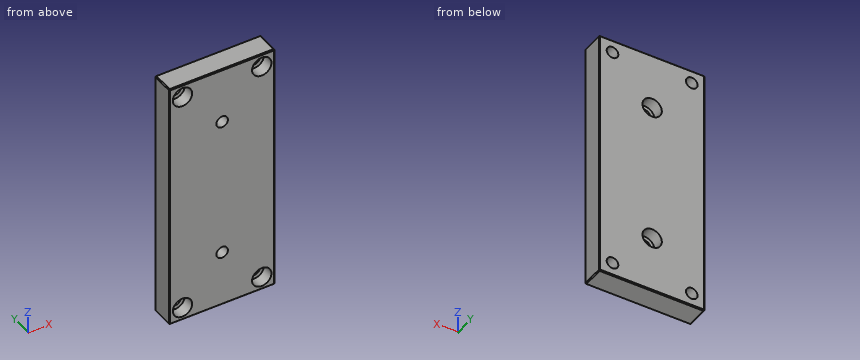
```python
from build123d import *

# Parameters (mm, degrees)
SKETCH_1_W                  = 60
SKETCH_1_H                  = 13
EXTRUDE_1_DEPTH             = 144
HOLE_WIZARD_2_D             = 6.6
HOLE_WIZARD_2_CBORE_D       = 11
HOLE_WIZARD_2_CBORE_DEPTH   = 6.8
CHAMFER_1_SIZE              = 0.5
HOLE_WIZARD_2_2_D           = 6.6
HOLE_WIZARD_2_2_CBORE_D     = 11
HOLE_WIZARD_2_2_CBORE_DEPTH = 6.8


with BuildPart() as part:
    # 草图1 → 凸台-拉伸1 (new body)
    with BuildSketch(Plane.XY):
        Rectangle(SKETCH_1_W, SKETCH_1_H)
    extrude(amount=EXTRUDE_1_DEPTH)

    # Hole Wizard 2 (through all)
    with Locations(Plane(origin=(0, 6.5, 0), x_dir=(1, 0, 0), z_dir=(0, 1, 0))):
        with Locations((0, -32), (0, -112)):
            CounterBoreHole(HOLE_WIZARD_2_D / 2, HOLE_WIZARD_2_CBORE_D / 2, HOLE_WIZARD_2_CBORE_DEPTH)

    # 倒角1
    chamfer_1_edges = [part.edges().sort_by_distance(p)[0] for p in [
        (-30, 0, 144),
        (0, -6.5, 144),
        (30, 0, 144),
        (0, -6.5, 0),
        (-30, 0, 0),
        (0, 6.5, 0),
        (30, 0, 0),
        (0, 6.5, 144),
        (30, -6.5, 72),
        (-30, -6.5, 72),
        (-30, 6.5, 72),
        (30, 6.5, 72),
    ]]
    chamfer(chamfer_1_edges, length=CHAMFER_1_SIZE)

    # Hole Wizard 2 2 (through all)
    with Locations(Plane(origin=(0, -6.5, 0), x_dir=(-1, 0, 0), z_dir=(0, -1, 0))):
        with Locations((-22.5, -136.5), (22.5, -136.5), (-22.5, -7.5), (22.5, -7.5)):
            CounterBoreHole(HOLE_WIZARD_2_2_D / 2, HOLE_WIZARD_2_2_CBORE_D / 2, HOLE_WIZARD_2_2_CBORE_DEPTH)


solid = part.part
```
Verification items for the finished model (mm, model axes). Coordinates: 2 decimals unless noted, no trailing zeros. Write each loop counter-clockwise with the first axis right and the second up, starting at its lowest first coordinate (ties: lowest second). Pieces come first, ordered by that corner, then holes. Notation, with made-up numbers: M 21,-23.5 L 30,-23.5 A31 cw 30,14.5 Z; hole C 26,-2.75 d8. An arc over 180 degrees is marked long. Answer as a JSON object with one key per item and string values. Group by question number.
(1) Gauge pin test, flat ends, axial feed: pin 1 (10 mm diameter, centred on x = 0, z = 112, fed in from +Y); pin 2 (5.5 mm diameter, centred on x = 21, z = 137.5, fed in from -Y). Record the tip position at first contact, or that the pin passes through.
(2) Cross-section at A-A, the plane z = 32. Record the cut outline in (x, y).
(3) Cross-section at B-B, the plane x = 22.5. Record the cut outline in (y, z), and give its area (3 significant figures).
(4) Material ranges on line 1 (Z direction, x = -22.5, y = -3.75); line 2 (X direction, y = -2.25, z = 136.5); line 3 (Z direction, x = 0, y = 2.5), recorded low to high.
(5) Cross-section at D-D, the plane z = 136.5. Record the cut outline in (x, y).
(6) Cross-section at C-C, the plane y = 4.25. Record the cut outline in (x, z), and give its area (3 significant figures).
Reply:
{
 "1": {"pin 1": "y = -0.3", "pin 2": "y = 0.3"},
 "2": {"outline": "M -30,-6 L -29.5,-6.5 L -3.3,-6.5 L -3.3,-0.3 L -5.5,-0.3 L -5.5,6.5 L -29.5,6.5 L -30,6 Z; M 3.3,-6.5 L 29.5,-6.5 L 30,-6 L 30,6 L 29.5,6.5 L 5.5,6.5 L 5.5,-0.3 L 3.3,-0.3 Z"},
 "3": {"outline": "M -6.5,0.5 L -6,0 L 6,0 L 6.5,0.5 L 6.5,4.2 L 0.3,4.2 L 0.3,2 L -6.5,2 Z; M -6.5,13 L 0.3,13 L 0.3,10.8 L 6.5,10.8 L 6.5,133.2 L 0.3,133.2 L 0.3,131 L -6.5,131 Z; M -6.5,142 L 0.3,142 L 0.3,139.8 L 6.5,139.8 L 6.5,143.5 L 6,144 L -6,144 L -6.5,143.5 Z", "area": "1,640 mm²"},
 "4": {"line 1": "0 to 2, 13 to 131, 142 to 144", "line 2": "-30 to -28, -17 to 17, 28 to 30", "line 3": "0 to 26.5, 37.5 to 106.5, 117.5 to 144"},
 "5": {"outline": "M -30,-6 L -29.5,-6.5 L -28,-6.5 L -28,0.3 L -25.8,0.3 L -25.8,6.5 L -29.5,6.5 L -30,6 Z; M -19.2,0.3 L -17,0.3 L -17,-6.5 L 17,-6.5 L 17,0.3 L 19.2,0.3 L 19.2,6.5 L -19.2,6.5 Z; M 25.8,0.3 L 28,0.3 L 28,-6.5 L 29.5,-6.5 L 30,-6 L 30,6 L 29.5,6.5 L 25.8,6.5 Z"},
 "6": {"outline": "M -30,0.5 L -29.5,0 L 29.5,0 L 30,0.5 L 30,143.5 L 29.5,144 L -29.5,144 L -30,143.5 Z; hole C -22.5,7.5 d6.6; hole C -22.5,136.5 d6.6; hole C 0,32 d11; hole C 0,112 d11; hole C 22.5,7.5 d6.6; hole C 22.5,136.5 d6.6", "area": "8,310 mm²"}
}
